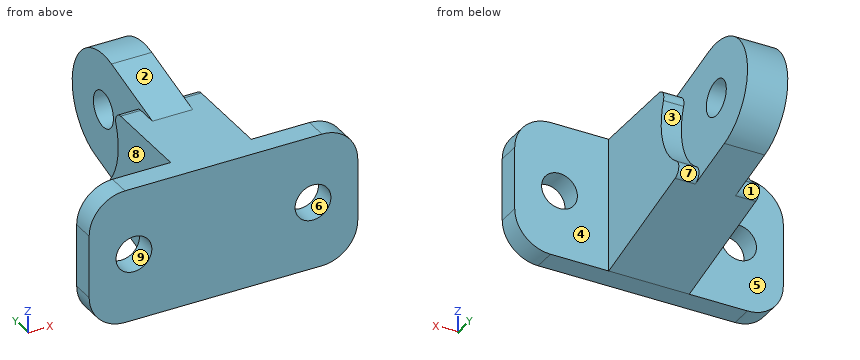
from build123d import *

# Parameters (mm, degrees)
BASE_PLATE_SKETCH_R       = 4
BASE_PLATE_DEPTH          = 5
TAPERED_UPRIGHT_DEPTH     = 9
PIVOT_LUG_DEPTH           = 10
LUG_SIDE_RELIEF_CUT_DEPTH = 5.5
PIVOT_BORE_SKETCH_R       = 4
PIVOT_BORE_8_DEPTH        = 66.873360759


with BuildPart() as part:
    # Base Plate Sketch → Base Plate (new body)
    with BuildSketch(Plane(origin=(0, 0, 0), x_dir=(1, 0, 0), z_dir=(0, 1, 0))):
        with BuildLine():
            Line((-22, 15), (22, 15))
            ThreePointArc((22, 15), (27.656854249, 12.656854249), (30, 7))
            Line((30, 7), (30, -7))
            ThreePointArc((30, -7), (27.656854249, -12.656854249), (22, -15))
            Line((22, -15), (-22, -15))
            ThreePointArc((-22, -15), (-27.656854249, -12.656854249), (-30, -7))
            Line((-30, -7), (-30, 7))
            ThreePointArc((-30, 7), (-27.656854249, 12.656854249), (-22, 15))
        make_face()
        with Locations(Location((-20, 0, 0), (0, 0, 270))):
            Circle(BASE_PLATE_SKETCH_R, mode=Mode.SUBTRACT)
        with Locations(Location((20, 0, 0), (0, 0, 270))):
            Circle(BASE_PLATE_SKETCH_R, mode=Mode.SUBTRACT)
    extrude(amount=BASE_PLATE_DEPTH)

    # Tapered Upright Sketch → Tapered Upright (add, symmetric)
    with BuildSketch(Plane(origin=(0, 0, 0), x_dir=(0, 0, -1), z_dir=(1, 0, 0))):
        with BuildLine():
            Line((-15, 20.368941598), (-15, 5))
            Line((-15, 5), (15, 5))
            Line((15, 5), (4.754898838, 43.235238064))
            ThreePointArc((4.754898838, 43.235238064), (-10.554412054, 52.074072829), (-19.393246819, 36.764761936))
            Line((-19.393246819, 36.764761936), (-15, 20.368941598))
        make_face()
    extrude(amount=TAPERED_UPRIGHT_DEPTH, both=True)

    # Pivot Lug Sketch → Pivot Lug (add, symmetric)
    with BuildSketch(Plane(origin=(0, 0, 0), x_dir=(0, 0, -1), z_dir=(1, 0, 0))):
        with BuildLine():
            Line((-15, 20.368941598), (-15, 25.04245288))
            ThreePointArc((-15, 25.04245288), (-14.135736214, 26.688692003), (-12.289896749, 26.91214627))
            ThreePointArc((-12.289896749, 26.91214627), (-3.083912061, 26.655991742), (4.289332839, 32.17423683))
            ThreePointArc((4.289332839, 32.17423683), (6.27753657, 33.028883618), (7.87954261, 31.573908753))
            Line((7.87954261, 31.573908753), (4.754898838, 43.235238064))
            ThreePointArc((4.754898838, 43.235238064), (-10.554412054, 52.074072829), (-19.393246819, 36.764761936))
            Line((-19.393246819, 36.764761936), (-15, 20.368941598))
        make_face()
    extrude(amount=PIVOT_LUG_DEPTH, both=True)

    # Lug Side Relief Sketch → Lug Side Relief Cut (cut)
    with BuildSketch(Plane(origin=(10, 0, 0), x_dir=(0, 0, -1), z_dir=(1, 0, 0))):
        with BuildLine():
            Line((-19.393246819, 36.764761936), (-15, 20.368941598))
            Line((-15, 20.368941598), (-15, 25.04245288))
            ThreePointArc((-15, 25.04245288), (-14.135736214, 26.688692003), (-12.289896749, 26.91214627))
            ThreePointArc((-12.289896749, 26.91214627), (-3.083912061, 26.655991742), (4.289332839, 32.17423683))
            ThreePointArc((4.289332839, 32.17423683), (6.27753657, 33.028883618), (7.87954261, 31.573908753))
            Line((7.87954261, 31.573908753), (4.754898838, 43.235238064))
            ThreePointArc((4.754898838, 43.235238064), (-10.554412054, 52.074072829), (-19.393246819, 36.764761936))
        make_face()
    lug_side_relief_cut = extrude(amount=-LUG_SIDE_RELIEF_CUT_DEPTH, mode=Mode.SUBTRACT)

    # Lug Side Relief Mirror: Lug Side Relief Cut across plane
    add(lug_side_relief_cut.mirror(Plane(origin=(0, 0, 0), x_dir=(0, 0, 1), z_dir=(1, 0, 0))), mode=Mode.SUBTRACT)

    # Pivot Bore Sketch → Pivot Bore Ø8 (cut, through all)
    with BuildSketch(Plane(origin=(4.5, 0, 0), x_dir=(0, 0, -1), z_dir=(1, 0, 0))):
        with Locations((-7.31917399, 40)):
            Circle(PIVOT_BORE_SKETCH_R)
    extrude(amount=-PIVOT_BORE_8_DEPTH, mode=Mode.SUBTRACT)


solid = part.part
Work out the finished part from the listing and answer in its coordinate system (mm). Face numbers are marked on the shaded views. A direction names the side the tool comes from. Give positions to 0.01 mm unless a question says otherwise; leave off trailing zeros. Write each loop counter-clockwise with the first axis right and the second up, starting at its lowest first coordinate (ties: lowest second). Pieces come first, ordered by that corner, then holes. Notation, with made-up numbers: (66, 5.25) - (80, 5.25) arc R23 cw to (80, 13.25) - close; hole circle Ø10 at (43.5, -37.75). An arc over 180 degrees is marked (long way). One line per item, written item: value. Start each with the question number.
1. Consider probe 1 along X at (y, z) = (2, 0); probe 2 along Y at (x, z) = (25, -14); probe 3 along X at (y, z) = (25, -7). Determine where each line is inside the solid, lowest interval first.
2. Find section B-B (y = 40). Write down the section's boundary in (x, z).
3. For the marked faces 1, 2, 3, 4 and 5, determine the directions among +Z, -Z, +X, -X, +Y, -Y from which every point of the face is accessible in a straight line to the end or side of a thin tool.
4. Find section D-D (z = -6). Write down the section's boundary in (x, y), then the cut area to 3 significant figures.
5. For a pull along X with two mould halves and no side action, classify the marked faces 6, 7, 8 and 9 as +X half, -X half, draft (parallel to the pull), parting line (faces both ways), or undercut.
6. Given pin 1 (6 mm diameter, centred on y = 16, z = -10, fed in from +X); pin 2 (8 mm diameter, centred on y = 20, z = -9, fed in from -X); pin 3 (10.5 mm diameter, centred on x = 16.5, z = 1, fed in from +Y), each flat-ended and moving along its own axis, determine where each tip first touches the part or whether it passes through.
7. Find section A-A (x = 17). Write down the section's boundary in (y, z), then the cut area to 3 significant figures.
8. Find section C-C (z = 0). Write down the section's boundary in (x, y).
Geometry results:
1. probe 1: -30 to -24, -16 to 16, 24 to 30
1. probe 2: 0 to 5
1. probe 3: -9 to 9
2. outline: (-4.5, -5.62) - (4.5, -5.62) - (4.5, 3.32) - (-4.5, 3.32) - close; (-4.5, 11.32) - (4.5, 11.32) - (4.5, 19.82) - (-4.5, 19.82) - close
3. face 1: -X, +Y
3. face 2: +Z, +X, -X, -Y
3. face 3: +X, +Y
3. face 4: +Z, -Z, +X, +Y
3. face 5: +Z, -Z, -X, +Y
4. outline: (-30, 0) - (30, 0) - (30, 5) - (9, 5) - (9, 33.06) - (4.5, 33.06) - (4.5, 38.59) - (-4.5, 38.59) - (-4.5, 33.06) - (-9, 33.06) - (-9, 5) - (-30, 5) - close
4. area: 855 mm2
5. face 6: undercut
5. face 7: draft
5. face 8: -X half
5. face 9: undercut
6. pin 1: x = 9
6. pin 2: x = -9
6. pin 3: y = 5
7. outline: (0, -15) - (5, -15) - (5, -2.65) - (0, -2.65) - close; (0, 2.65) - (5, 2.65) - (5, 15) - (0, 15) - close
7. area: 124 mm2
8. outline: (-30, 0) - (-24, 0) - (-24, 5) - (-30, 5) - close; (-16, 0) - (16, 0) - (16, 5) - (9, 5) - (9, 28.07) - (4.5, 28.07) - (4.5, 50.13) - (-4.5, 50.13) - (-4.5, 28.07) - (-9, 28.07) - (-9, 5) - (-16, 5) - close; (24, 0) - (30, 0) - (30, 5) - (24, 5) - close
